Read the model definition and answer for the solid it produces. Units are mm, in the model's axes. Face numbers are marked on the shaded views. Give positions to 0.01 mm unless a question says otherwise; leave off trailing zeros. Loops run counter-clockwise (first coordinate to the right, second up) from the corner with the lowest first, then second, coordinate; pieces in that order, holes last. Notation, with made-up numbers: (50, 49) - (59, 49) arc R17 ccw to (59, 55) - close; hole circle Ø10 at (4.25, 48). An arc over 180 degrees is marked (long way). Use a Markdown table: item, result. Add a question column.
Item 1: This flat-tipped pin is pushed along its axis until it touches: P1, Ø6, axis at x = 2, z = 0, coming from the -Y side. Where does it stop, or does it pass through?
Item 2: A cutting plane is placed at B-B (x = 0). Determine the outline of the cut face in (y, z).
Item 3: Consider probe 1 along X at (y, z) = (4.8, 0); probe 2 along Y at (x, z) = (-6.5, -9.5); probe 3 along X at (y, z) = (1, 11). Determine where each line is inside the solid, lowest interval first. Write a range as [from, to].
Item 4: A cutting plane is placed at A-A (z = 0). Determine the outline of the cut face in (x, y), plus the area to 3 significant figures.
Item 5: A cutting plane is placed at C-C (y = 5.75). Determine the outline of the cut face in (x, z).
Item 6: A cutting plane is placed at D-D (x = 12.5). Determine the outline of the cut face in (y, z).
Item 7: For a pull along Z with two mould halves and no side action, classify the marked faces 1, 2 and 3 as +Z half, -Z half, draft (parallel to the pull), parting line (faces both ways), or undercut.
from build123d import *

# Parameters (mm, degrees)
SKETCH1_W           = 40
SKETCH1_H           = 40
BOSS_EXTRUDE1_DEPTH = 8
CHAMFER1_SIZE       = 1
SKETCH2_R           = 15.5
CUT_EXTRUDE1_DEPTH  = 3.5
SKETCH3_R           = 4.25
CUT_EXTRUDE2_DEPTH  = 30.393876913
SKETCH4_R           = 2.15
CUT_EXTRUDE3_DEPTH  = 10


with BuildPart() as part:
    # Sketch1 → Boss-Extrude1 (new body)
    with BuildSketch(Plane(origin=(0, 0, 0), x_dir=(1, 0, 0), z_dir=(0, 1, 0))):
        Rectangle(SKETCH1_W, SKETCH1_H)
    extrude(amount=BOSS_EXTRUDE1_DEPTH)

    # Chamfer1
    chamfer1_edges = [part.edges().sort_by_distance(p)[0] for p in [
        (20, 4, 20),
        (-20, 4, 20),
        (-20, 4, -20),
        (20, 4, -20),
    ]]
    chamfer(chamfer1_edges, length=CHAMFER1_SIZE)

    # Sketch2 → Cut-Extrude1 (cut)
    with BuildSketch(Plane.XZ):
        with Locations(Location((0, 0, 0), (0, 0, 270))):
            Circle(SKETCH2_R)
    extrude(amount=-CUT_EXTRUDE1_DEPTH, mode=Mode.SUBTRACT)

    # Sketch3 → Cut-Extrude2 (cut, through all)
    with BuildSketch(Plane(origin=(0, 8, 0), x_dir=(1, 0, 0), z_dir=(0, 1, 0))):
        with Locations(Location((0, 0, 0), (0, 0, 270))):
            Circle(SKETCH3_R)
    extrude(amount=-CUT_EXTRUDE2_DEPTH, mode=Mode.SUBTRACT)

    # Sketch4 → Cut-Extrude3 (cut)
    with BuildSketch(Plane.XZ):
        with Locations(Location((16.263455967, 16.263455967, 0), (0, 0, 270))):
            Circle(SKETCH4_R)
        with Locations(Location((-16.263455967, -16.263455967, 0), (0, 0, 270))):
            Circle(SKETCH4_R)
    extrude(amount=-CUT_EXTRUDE3_DEPTH, mode=Mode.SUBTRACT)


solid = part.part
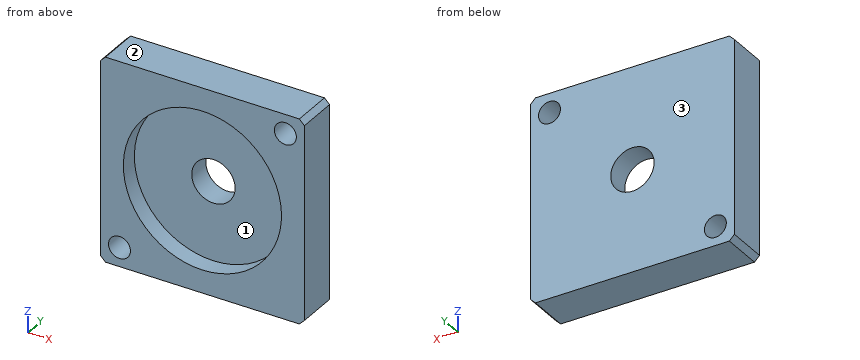
Geometry says:
| question | item | result |
|---|---|---|
| 1 | P1 | y = 3.5 |
| 2 | outline | (0, -20) - (8, -20) - (8, -4.25) - (3.5, -4.25) - (3.5, -15.5) - (0, -15.5) - close; (0, 15.5) - (3.5, 15.5) - (3.5, 4.25) - (8, 4.25) - (8, 20) - (0, 20) - close |
| 3 | probe 1 | [-20, -4.25], [4.25, 20] |
| 3 | probe 2 | [3.5, 8] |
| 3 | probe 3 | [-20, -10.92], [10.92, 20] |
| 4 | outline | (-20, 0) - (-15.5, 0) - (-15.5, 3.5) - (-4.25, 3.5) - (-4.25, 8) - (-20, 8) - close; (4.25, 3.5) - (15.5, 3.5) - (15.5, 0) - (20, 0) - (20, 8) - (4.25, 8) - close |
| 4 | area | 173 mm² |
| 5 | outline | (-20, -19) - (-19, -20) - (19, -20) - (20, -19) - (20, 19) - (19, 20) - (-19, 20) - (-20, 19) - close; hole circle Ø4.3 at (-16.26, -16.26); hole circle Ø8.5 at (0, 0); hole circle Ø4.3 at (16.26, 16.26) |
| 6 | outline | (0, -20) - (8, -20) - (8, 20) - (0, 20) - (0, 9.17) - (3.5, 9.17) - (3.5, -9.17) - (0, -9.17) - close |
| 7 | face 1 | undercut |
| 7 | face 2 | +Z half |
| 7 | face 3 | draft |
